from build123d import *

# Parameters (mm, degrees)
BOSS_EXTRUDE1_DEPTH      = 2
BOSS_EXTRUDE1_DEPTH_BACK = 2
SKETCH1_R                = 7.5
SKETCH1_R_2              = 5
SKETCH2_R                = 7.1
SKETCH2_R_2              = 5.605
CUT_EXTRUDE1_DEPTH       = 0.5


with BuildPart() as part:
    # Sketch1 → Boss-Extrude1 (new, two sides: drawn at the far end of the back side and taken through both)
    with BuildSketch(Plane.XY.offset(-BOSS_EXTRUDE1_DEPTH_BACK)):
        Circle(SKETCH1_R)
        Circle(SKETCH1_R_2, mode=Mode.SUBTRACT)
    extrude(amount=BOSS_EXTRUDE1_DEPTH + BOSS_EXTRUDE1_DEPTH_BACK)

    # Sketch2 → Cut-Extrude1 (cut)
    with BuildSketch(Plane.XY.offset(2)):
        Circle(SKETCH2_R)
        Circle(SKETCH2_R_2, mode=Mode.SUBTRACT)
    cut_extrude1 = extrude(amount=-CUT_EXTRUDE1_DEPTH, mode=Mode.SUBTRACT)

    # Mirror1: Cut-Extrude1 across plane
    add(cut_extrude1.mirror(Plane.XY), mode=Mode.SUBTRACT)


solid = part.part
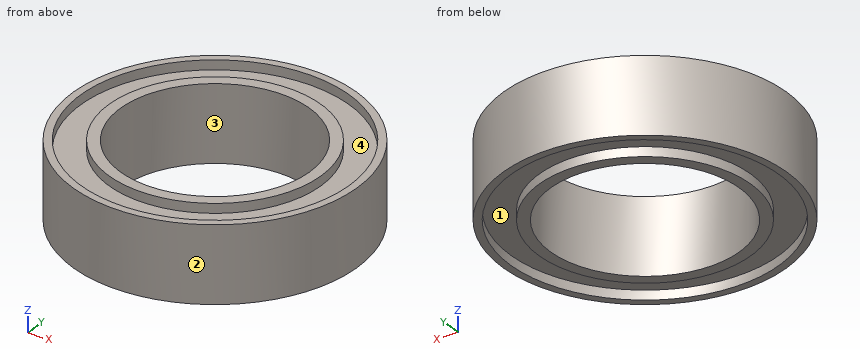
The listing builds one solid part. Answer for the finished solid, in the listing's coordinates (mm). Face numbers are marked on the shaded views. A direction names the side the tool comes from. Coordinates: 2 decimals unless noted, no trailing zeros. Write each loop counter-clockwise with the first axis right and the second up, starting at its lowest first coordinate (ties: lowest second). Pieces come first, ordered by that corner, then holes. Notation, with made-up numbers: M 41,4.25 L 56,4.25 A22 cw 56,26.25 Z; hole C -27,2 d10. An arc over 180 degrees is marked long. Use one line per item in the form item = value.
Item 1: Given P1, Ø4, axis at x = -5.5, y = 4, coming from the -Z side; P2, Ø1, axis at y = 2.5, z = 1, coming from the -X side, each flat-ended and moving along its own axis, determine where each tip first touches the part or whether it passes through.
Model answer:
P1 = -2
P2 = -7.23
Item 2: Find section D-D, the plane x = 6.5. Give the vertices of the cut face in (y, z), plus the area to 3 significant figures.
Model answer:
outline = M -3.74,-2 L -2.86,-2 L -2.86,-1.5 L 2.86,-1.5 L 2.86,-2 L 3.74,-2 L 3.74,2 L 2.86,2 L 2.86,1.5 L -2.86,1.5 L -2.86,2 L -3.74,2 Z
area = 24.2 mm2
Item 3: Find section C-C, the plane z = 0.4. Give the vertices of the cut face in (x, y), plus the area to 3 significant figures.
Model answer:
outline = C 0,0 d15; hole C 0,0 d10
area = 98.2 mm2
Item 4: Find the intervals of material crossed by probe 1 along Y at (x, z) = (0, -1.6) (3 decimals); probe 2 along Y at (x, z) = (0, -0.15); probe 3 along X at (y, z) = (-2.5, -1.7), in increasing order.
Model answer:
probe_1 = -7.5 to -7.1, -5.605 to -5, 5 to 5.605, 7.1 to 7.5
probe_2 = -7.5 to -5, 5 to 7.5
probe_3 = -7.07 to -6.65, -5.02 to -4.33, 4.33 to 5.02, 6.65 to 7.07
Item 5: Find section A-A, the plane y = 0. Give the vertices of the cut face in (x, z) (3 decimals), plus the area to 3 significant figures.
Model answer:
outline = M -7.5,-2 L -7.1,-2 L -7.1,-1.5 L -5.605,-1.5 L -5.605,-2 L -5,-2 L -5,2 L -5.605,2 L -5.605,1.5 L -7.1,1.5 L -7.1,2 L -7.5,2 Z; M 5,-2 L 5.605,-2 L 5.605,-1.5 L 7.1,-1.5 L 7.1,-2 L 7.5,-2 L 7.5,2 L 7.1,2 L 7.1,1.5 L 5.605,1.5 L 5.605,2 L 5,2 Z
area = 17.0 mm2
Item 6: For the marked faces 3 and 4, determine the directions among +Z, -Z, +X, -X, +Y, -Y from which every point of the face is accessible in a straight line to the end or side of a thin tool.
Model answer:
face_3 = +Z, -Z
face_4 = +Z
Item 7: The mould has two halves that part along X. Classify the marked faces 1 and 2: released by +X, released by -X, zero draft, split by the parting line, or undercut.
Model answer:
face_1 = undercut
face_2 = split by the parting line
